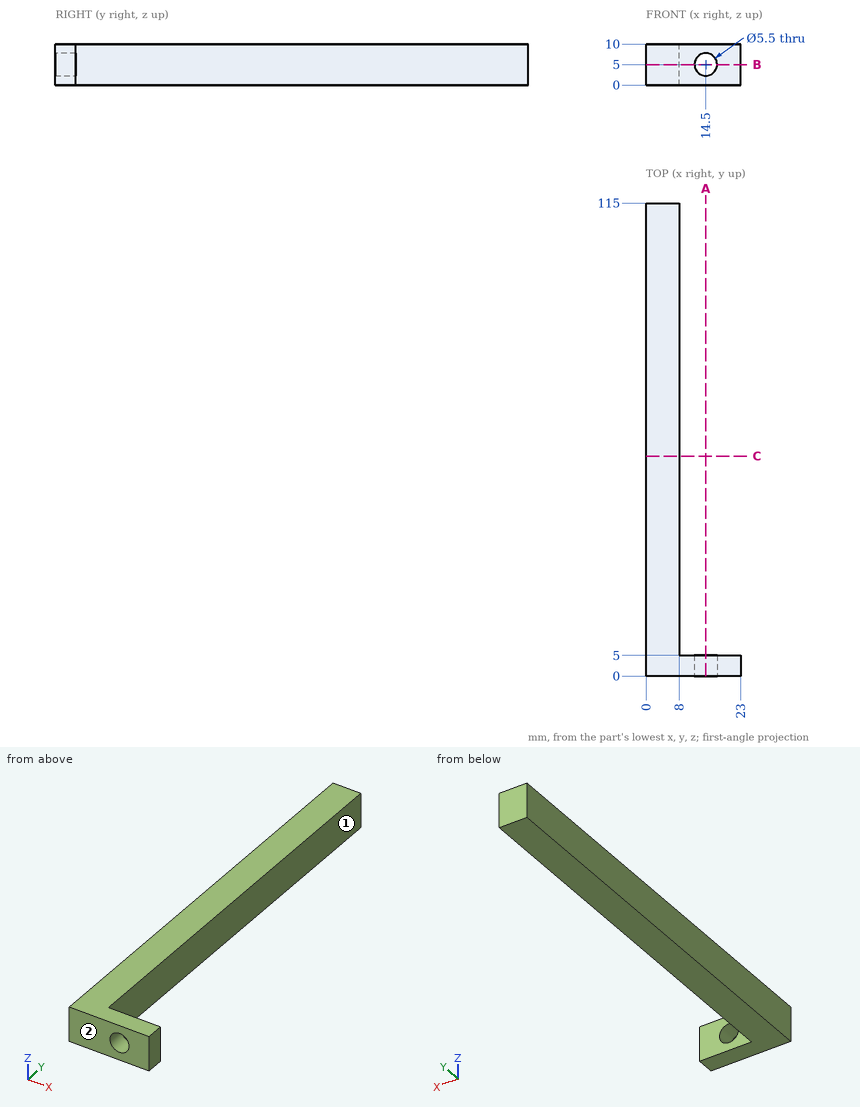
Check sheet for the drawn part. Datum: minimum x, y, z corner. Units: mm. A direction names the side the tool comes from. Give positions to 0.01 mm unless a question says otherwise; leave off trailing zeros. Loops run counter-clockwise (first coordinate to the right, second up) from the corner with the lowest first, then second, coordinate; pieces in that order, holes last. Notation, with made-up numbers: M 34,-3 L 88,-3 A30 ccw 88,29 Z; hole C -25,89 d10. An arc over 180 degrees is marked long. Return JSON: item names as keys, results as strings.
1) Section check A-A, the plane x = 14.5. Enter the section's corners in (y, z), and give its area (3 significant figures).
Findings:
{"outline": "M 0,0 L 5,0 L 5,2.25 L 0,2.25 Z; M 0,7.75 L 5,7.75 L 5,10 L 0,10 Z", "area": "22.5 mm2"}
2) Material ranges on L1, parallel to X at y = 1.5, z = 5; L2, parallel to X at y = 92, z = 5.75; L3, parallel to Y at x = 15.75, z = 9.5, recorded low to high. Write a range as [from, to].
Findings:
{"L1": "x = [0, 11.75], [17.25, 23]", "L2": "x = [0, 8]", "L3": "y = [0, 5]"}
3) Tool access check on the marked faces 1 and 2. Record the directions out of +Z, -Z, +X, -X, +Y, -Y that give a thin tool (end or side, any length) a straight path to the whole face; none if there is none.
Findings:
{"face 1": "+Z, -Z, +X, +Y", "face 2": "+Z, -Z, +X, -X, -Y"}
4) Gauge pin test, flat ends, axial feed: P1, Ø5, axis at x = 17.5, z = 7, coming from the +Y side; P2, Ø5, axis at y = 75, z = 4, coming from the +X side. Record the tip position at first contact, or that the pin passes through.
Findings:
{"P1": "stops at y = 5", "P2": "stops at x = 8"}
5) Section check C-C, the plane y = 53.5. Enter the section's corners in (x, z), and give its area (3 significant figures).
Findings:
{"outline": "M 0,0 L 8,0 L 8,10 L 0,10 Z", "area": "80.0 mm2"}
6) Section check B-B, the plane z = 5. Enter the section's corners in (x, y), and give its area (4 significant figures).
Findings:
{"outline": "M 0,0 L 11.75,0 L 11.75,5 L 8,5 L 8,115 L 0,115 Z; M 17.25,0 L 23,0 L 23,5 L 17.25,5 Z", "area": "967.5 mm2"}
